The model under review builds one solid part; all positions refer to its coordinate system, in mm. A direction names the side the tool comes from. Round coordinates to 2 decimals unless told otherwise and drop trailing zeros. Write each loop counter-clockwise with the first axis right and the second up, starting at its lowest first coordinate (ties: lowest second). Pieces come first, ordered by that corner, then holes. Notation, with made-up numbers: M 59.5,0 L 94.5,0 A10 cw 94.5,18 Z; hole C 80,-29.75 d3. An arc over 180 degrees is marked long. One line per item, written item: value. Start each with the question number.
1) Take a section at D-D, the plane y = 487. Write out the cut boundary in (x, z).
2) Take a section at A-A, the plane x = 176. Write out the cut boundary in (y, z).
3) Tool access review of faces 1 (the face through (170.607, 175.872, 7.888)), 2 (the face through (40.28, 325.56, 7.89)): name each direction out of +Z, -Z, +X, -X, +Y, -Y from which nothing blocks a thin tool from reaching the whole face with its end or side.
4) Mouldability with a two-part tool opening along Y and no side actions: class faces 3 (the face through (79.85, 74.83, 7.89)), 4 (the face through (165, 85, 8)), 5 (the face through (38, 416, 8)) as +Y half, -Y half, draft (parallel to the pull), parting line (faces both ways), or undercut.
5) Take a section at B-B, the plane z = 11.75. Write out the cut boundary in (x, y).
6) Take a section at C-C, the plane x = 322.5. Write out the cut boundary in (y, z), and give its area (3 significant figures).
7) For P1, Ø3, axis at x = 363, z = 5.5, coming from the -Y side; P2, Ø4, axis at y = 232, z = 10.5, coming from the +X side; P3, Ø5, axis at y = 432.5, z = 5, coming from the +X side, all flat-tipped, find the tip position at first contact; note any pin that passes through.
8) Wall thickness on probe 1 along Y at (x, z) = (353.5, 5.5); probe 2 along X at (y, z) = (454, 11); probe 3 along Y at (x, z) = (57, 10.5) (3 decimals): over which ranges is each line inside the solid? List them lowest first.
from build123d import *

# Parameters (mm, degrees)
BOSS_EXTRUDE1_DEPTH = 16


with BuildPart() as part:
    # Sketch1 → Boss-Extrude1 (new body)
    with BuildSketch(Plane.XY):
        with BuildLine():
            Line((0, 145), (0, 563))
            Line((0, 563), (10, 573))
            Line((10, 573), (550, 573))
            ThreePointArc((550, 573), (557.071067812, 570.071067812), (560, 563))
            Line((560, 563), (560, 524))
            Line((560, 524), (68, 524))
            ThreePointArc((68, 524), (46.786796564, 515.213203436), (38, 494))
            Line((38, 494), (38, 334.829857024))
            ThreePointArc((38, 334.829857024), (40.33946289, 325.443407802), (46.8105429, 318.252883543))
            Line((46.8105429, 318.252883543), (222, 200))
            Line((222, 200), (184.847185197, 186.638022746))
            ThreePointArc((184.847185197, 186.638022746), (170.458357389, 175.662455442), (165, 158.408245001))
            Line((165, 158.408245001), (165, 10))
            Line((165, 10), (157.488351016, 6.601146077))
            Line((157.488351016, 6.601146077), (0, 145))
        make_face()
    extrude(amount=BOSS_EXTRUDE1_DEPTH)


solid = part.part
Checked values:
1. outline: M 0,0 L 38,0 L 38,16 L 0,16 Z
2. outline: M 181.62,0 L 231.05,0 L 231.05,16 L 181.62,16 Z; M 524,0 L 573,0 L 573,16 L 524,16 Z
3. face 1: +Z, -Z, +X, -Y
3. face 2: +Z, -Z, +X
4. face 3: -Y half
4. face 4: draft
4. face 5: undercut
5. outline: M 0,145 L 157.49,6.6 L 165,10 L 165,158.41 A30 cw 184.85,186.64 L 222,200 L 46.81,318.25 A20 cw 38,334.83 L 38,494 A30 cw 68,524 L 560,524 L 560,563 A10 ccw 550,573 L 10,573 L 0,563 Z
6. outline: M 524,0 L 573,0 L 573,16 L 524,16 Z
6. area: 784 mm2
7. P1: stops at y = 524
7. P2: stops at x = 177.56
7. P3: stops at x = 38
8. probe 1: y = 524 to 573
8. probe 2: x = 0 to 38
8. probe 3: y = 94.909 to 311.375, 521.911 to 573
